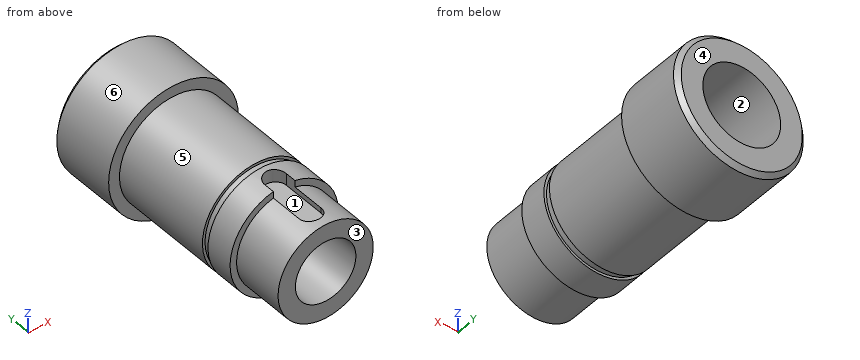
```python
from build123d import *

# Parameters (mm, degrees)
SKETCH2_W          = 4.874466188
SKETCH2_H          = 1.6
SKETCH3_R          = 9
CUT_EXTRUDE1_DEPTH = 20
M16_TAPPED_HOLE2_D = 14
CHAMFER1_SIZE      = 1
CUT_EXTRUDE2_START = 12.5
CUT_EXTRUDE2_DEPTH = 3
SKETCH10_R         = 15
SKETCH10_R_2       = 11
CUT_EXTRUDE3_DEPTH = 12


with BuildPart() as part:
    # Sketch1 → Revolve1 (revolve)
    with BuildSketch(Plane.XY, mode=Mode.PRIVATE) as revolve1_sk:
        Polygon((6, 60), (15, 60), (15, 44), (12.5, 44), (12.5, 0), (6, 0), align=None)
    revolve(revolve1_sk.sketch.rotate(Axis((0, 0, 0), (0, 1, 0)), 90), axis=Axis((0, 0, 0), (0, 1, 0)))

    # Sketch2 → Cut-Revolve1 (revolve, cut)
    with BuildSketch(Plane.XY, mode=Mode.PRIVATE) as cut_revolve1_sk:
        with Locations((-14.337233094, 19.2)):
            Rectangle(SKETCH2_W, SKETCH2_H)
    revolve(cut_revolve1_sk.sketch.rotate(Axis((0, 0, 0), (0, 1, 0)), 270), axis=Axis((0, 0, 0), (0, 1, 0)), mode=Mode.SUBTRACT)

    # Sketch3 → Cut-Extrude1 (cut)
    with BuildSketch(Plane(origin=(0, 60, 0), x_dir=(1, 0, 0), z_dir=(0, 1, 0))):
        with Locations(Location((0, 0, 0), (0, 0, 270))):
            Circle(SKETCH3_R)
    extrude(amount=-CUT_EXTRUDE1_DEPTH, mode=Mode.SUBTRACT)

    # M16 Tapped Hole2 (through all)
    with Locations(Plane(origin=(0, 0, 0), x_dir=(-1, 0, 0), z_dir=(0, -1, 0))):
        with Locations((0, 0)):
            Hole(M16_TAPPED_HOLE2_D / 2)

    # Chamfer1
    chamfer1_edges = [part.edges().sort_by_distance(p)[0] for p in [
        (0, 0, 12.5),
        (0, 60, 15),
    ]]
    chamfer(chamfer1_edges, length=CHAMFER1_SIZE)

    # Sketch8 → Cut-Extrude2 (cut)
    with BuildSketch(Plane.XY.offset(CUT_EXTRUDE2_START)):
        with BuildLine():
            Line((2.5, 14.5), (2.5, 4.5))
            ThreePointArc((2.5, 4.5), (0, 2), (-2.5, 4.5))
            Line((-2.5, 4.5), (-2.5, 14.5))
            ThreePointArc((-2.5, 14.5), (0, 17), (2.5, 14.5))
        make_face()
    extrude(amount=-CUT_EXTRUDE2_DEPTH, mode=Mode.SUBTRACT)

    # Sketch10 → Cut-Extrude3 (cut)
    with BuildSketch(Plane.XZ):
        with Locations(Location((0, 0, 0), (0, 0, 270))):
            Circle(SKETCH10_R)
        with Locations(Location((0, 0, 0), (0, 0, 270))):
            Circle(SKETCH10_R_2, mode=Mode.SUBTRACT)
    extrude(amount=-CUT_EXTRUDE3_DEPTH, mode=Mode.SUBTRACT)


solid = part.part
```
The model under review builds one solid part; all positions refer to its coordinate system, in mm. Face numbers are marked on the shaded views. A direction names the side the tool comes from. Round coordinates to 2 decimals unless told otherwise and drop trailing zeros. Loops run counter-clockwise (first coordinate to the right, second up) from the corner with the lowest first, then second, coordinate; pieces in that order, holes last.
Item 1: For line 1 (X direction, y = 47.75, z = 0); line 2 (Y direction, x = -10.25, z = -7); line 3 (Y direction, x = -1.5, z = -13), list the stretches that pass through material, from the lowest coordinate up.
Determined:
line 1: x = -15 to -9, 9 to 15
line 2: y = 12 to 18.4, 20 to 60
line 3: y = 44 to 60
Item 2: For the marked faces 5 and 6, list the 3-axis set-ups (+Z, -Z, +X, -X, +Y, -Y) from which the entire face can be reached by the end or side of a thin tool; tool diameter is ignored.
Determined:
face 5: -Y
face 6: +Y, -Y
Item 3: Clearance check with flat-ended pins moving along their axes: pin 1 Ø1 at (y, z) = (48.5, -9.5) entering from +X; pin 2 Ø7.5 at (x, z) = (4.5, 5.5) entering from +Y; pin 3 Ø8 at (y, z) = (46.5, -10) entering from +X; pin 4 Ø8 at (x, y) = (9.5, 27.5) entering from +Z (3 decimals). State where each tip first meets the part, or that it passes through.
Determined:
pin 1: stops at x = 12
pin 2: stops at y = 60
pin 3: stops at x = 13.75
pin 4: stops at z = 11.225
Item 4: Take a section at D-D (y = 9). Write out the cut boundary in (x, z), then the cut area to 3 significant figures.
Determined:
outline: (-2.5, 9.5) - (-2.5, 10.71) arc R11 ccw (long way) to (2.5, 10.71) - (2.5, 9.5) - close; hole circle Ø14 at (0, 0)
area: 219 mm2
Item 5: Take a section at C-C (y = 41). Write out the cut boundary in (x, z), then the cut area to 3 significant figures.
Determined:
outline: circle Ø25 at (0, 0); hole circle Ø18 at (0, 0)
area: 236 mm2
Item 6: Mouldability with a two-part tool opening along Y and no side actions: class the marked faces 1, 2, 3 and 4 as released by +Y, released by -Y, zero draft, split by the parting line, or undercut.
Determined:
face 1: undercut
face 2: zero draft
face 3: released by -Y
face 4: released by +Y
